Verification items for this drawing (mm, ordinates from the low corner). A direction names the side the tool comes from. Give positions to 0.01 mm unless a question says otherwise; leave off trailing zeros. Loops run counter-clockwise (first coordinate to the right, second up) from the corner with the lowest first, then second, coordinate; pieces in that order, holes last. Notation, with made-up numbers: (-11, 89) -> (39, 89) arc R18 ccw to (39, 120) -> close; hole circle Ø4 at (55.25, 0). An arc over 180 degrees is marked (long way). Answer as CSV lines item,"result". Start each with the question number.
(1) Access from +Z, -Z, +X, -X, +Y, -Y to the whole of each face (thin tool, end or side, straight path). Record for the marked faces 1 and 2.
(2) Section check A-A on y = 20. Enter the section's corners in (x, z), plus the area to 3 significant figures.
(3) Gauge pin test, flat ends, axial feed: pin 1 Ø3 at (y, z) = (7.5, 60.5) entering from -X; pin 2 Ø4 at (y, z) = (10, 18) entering from -X; pin 3 Ø1 at (y, z) = (17.5, 62.5) entering from -X. Record the tip position at first contact, or that the pin passes through.
(4) Section check C-C on z = 50. Enter the section's corners in (x, y).
(5) Section check B-B on x = 20. Enter the section's corners in (y, z), plus the area to 3 significant figures.
(6) Material ranges on line 1 (X direction, y = 20.5, z = 31); line 2 (Z direction, x = 6.5, y = 26); line 3 (Z direction, x = 12, y = 35), recorded low to high. Write a range as from..to.
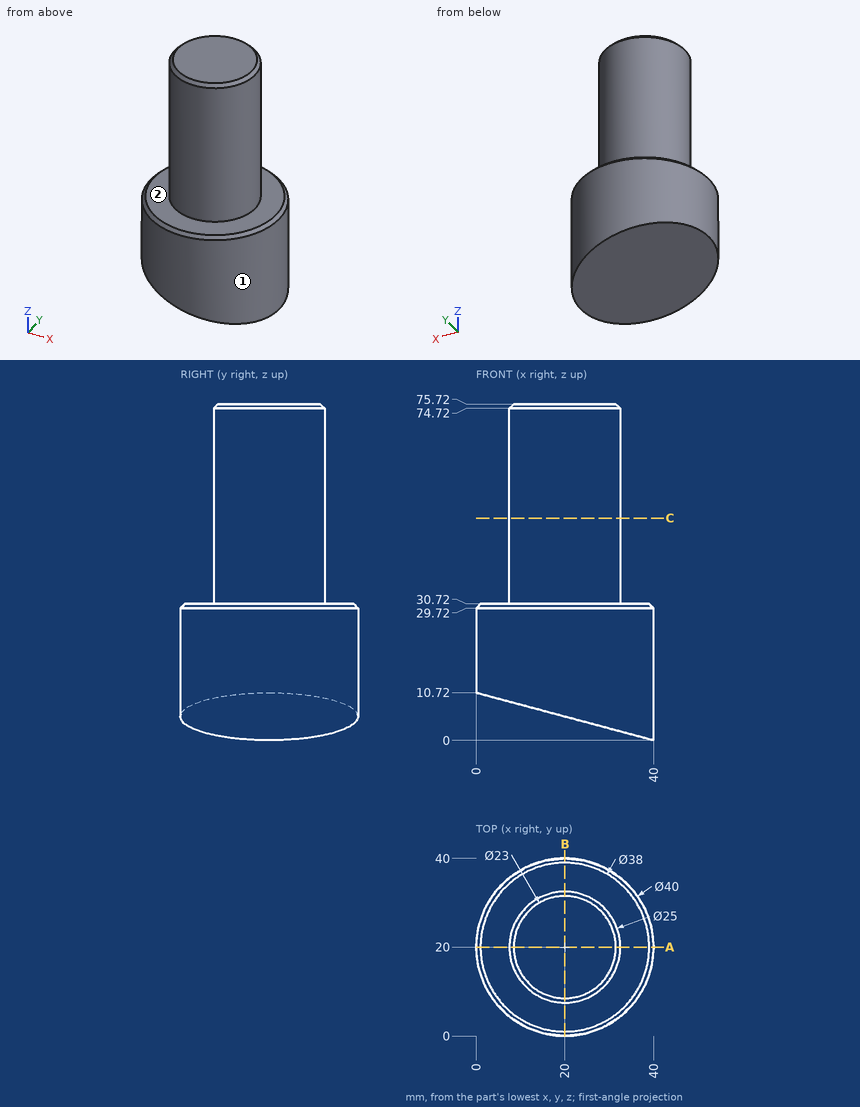
Working result:
1,face 1,"+Z, -Z"
1,face 2,"+Z"
2,outline,"(0, 10.72) -> (40, 0) -> (40, 29.72) -> (39, 30.72) -> (32.5, 30.72) -> (32.5, 74.72) -> (31.5, 75.72) -> (8.5, 75.72) -> (7.5, 74.72) -> (7.5, 30.72) -> (1, 30.72) -> (0, 29.72) -> close"
2,area,"2,140 mm^2"
3,pin 1,"stops at x = 14.06"
3,pin 2,"stops at x = 1.67"
3,pin 3,"stops at x = 7.66"
4,outline,"circle Ø25 at (20, 20)"
5,outline,"(0, 5.36) -> (40, 5.36) -> (40, 29.72) -> (39, 30.72) -> (32.5, 30.72) -> (32.5, 74.72) -> (31.5, 75.72) -> (8.5, 75.72) -> (7.5, 74.72) -> (7.5, 30.72) -> (1, 30.72) -> (0, 29.72) -> close"
5,area,"2,140 mm^2"
6,line 1,"x = 7.51..32.49"
6,line 2,"z = 8.98..30.72"
6,line 3,"z = 7.5..30.72"
